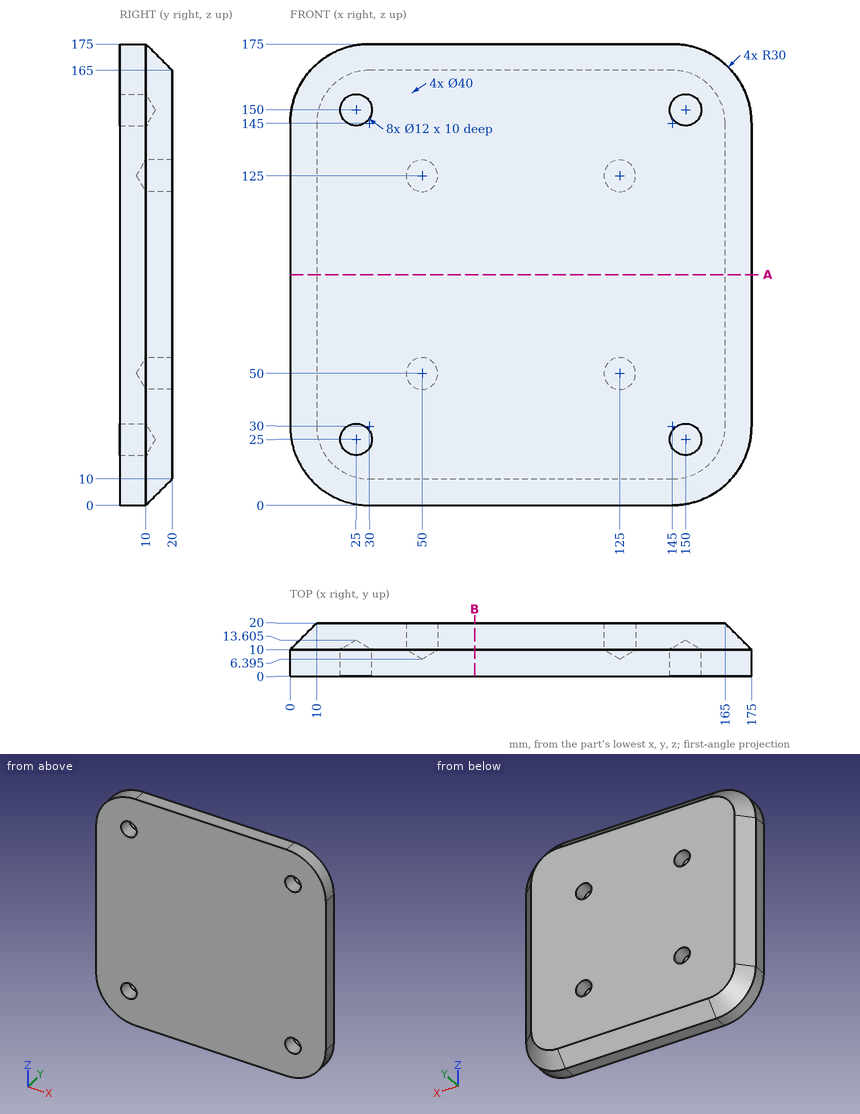
Source: three-view drawing plus pictorial views. Frame: mm from the lowest corner of the part. Give positions to 0.01 mm unless a question says otherwise; leave off trailing zeros. Order: outer loops, then holes, each group sorted by start corner. A loop starts at its lowest first (then second) coordinate and runs counter-clockwise, first axis right, second up. Notation, with made-up numbers: (18, 4.25) - (60, 4.25) arc R27 cw to (60, 43.25) - close; hole circle Ø11 at (14.5, 45.25). An arc over 180 degrees is marked (long way). Answer as a JSON object with one key per item and string values. Group by question number.
Q1. First-contact query: pin 1 Ø3 at (x, y) = (149.5, 9.5) entering from -Z; pin 2 Ø3 at (y, z) = (13, 26.5) entering from +X (1 decimal); pin 3 Ø9.5 at (x, z) = (50, 50) entering from +Y. Flat tips, straight axial feed; report the tip coordinate or a pass-through.
Q2. Line query: probe 1 along Z at (x, y) = (150, 3.25); probe 2 along Z at (x, y) = (50, 14); probe 3 along X at (y, z) = (4, 21). Output: solid intervals per line, ascending.
Q3. Cut plane B-B, the plane x = 70. Output: boundary loops of the cut face in (y, z), then the cut area to 3 significant figures.
Q4. Cut plane A-A, the plane z = 87.5. Output: boundary loops of the cut face in (x, y), then the cut area to 3 significant figures.
Results:
{
 "1": {"pin 1": "z = 0.15", "pin 2": "x = 173.3", "pin 3": "y = 9.25"},
 "2": {"probe 1": "0.42 to 19, 31 to 144, 156 to 174.58", "probe 2": "4 to 44, 56 to 119, 131 to 171", "probe 3": "1.38 to 20.53, 29.47 to 145.53, 154.47 to 173.62"},
 "3": {"outline": "(0, 0) - (10, 0) - (20, 10) - (20, 165) - (10, 175) - (0, 175) - close", "area": "3,400 mm^2"},
 "4": {"outline": "(0, 0) - (175, 0) - (175, 10) - (165, 20) - (10, 20) - (0, 10) - close", "area": "3,400 mm^2"}
}
